```python
from build123d import *

# Parameters (mm, degrees)
SKETCH1_R           = 20
SKETCH1_R_2         = 12.5
BOSS_EXTRUDE1_DEPTH = 112
CHAMFER1_SIZE       = 1


with BuildPart() as part:
    # Sketch1 → Boss-Extrude1 (new body)
    with BuildSketch(Plane(origin=(0, 0, 0), x_dir=(1, 0, 0), z_dir=(0, 1, 0))):
        with Locations(Location((0, 0, 0), (0, 0, 270))):
            Circle(SKETCH1_R)
        with Locations(Location((0, 0, 0), (0, 0, 270))):
            Circle(SKETCH1_R_2, mode=Mode.SUBTRACT)
    extrude(amount=BOSS_EXTRUDE1_DEPTH)

    # Chamfer1
    chamfer1_edges = [part.edges().sort_by_distance(p)[0] for p in [
        (0, 0, -20),
        (0, 112, -20),
        (0, 0, -12.5),
        (0, 112, -12.5),
    ]]
    chamfer(chamfer1_edges, length=CHAMFER1_SIZE)


solid = part.part
```
Source: CAD feature listing. Evaluate the final solid. Frame: model axes, mm. Give positions to 0.01 mm unless a question says otherwise; leave off trailing zeros. Write each loop counter-clockwise with the first axis right and the second up, starting at its lowest first coordinate (ties: lowest second). Pieces come first, ordered by that corner, then holes.
1. Section query B-B (x = 0). Return the cut outline in (y, z).
2. Section query C-C (y = 67). Return the cut outline in (x, z), then the cut area to 3 significant figures.
3. Pull-direction query (Z, two-part tool) for faces 1 (the face through (3.755, 55.23, 11.923)), 2 (the face through (-19.524, 55.23, -4.336)), 3 (the face through (12.9, 112, -4.5)); classes: +Z half, -Z half, draft (parallel to the pull), parting line (faces both ways), or undercut.
4. First-contact query: pin 1 (3 mm diameter, centred on y = 55.5, z = 5, fed in from -X); pin 2 (12 mm diameter, centred on x = 4.5, z = -12, fed in from +Y); pin 3 (10 mm diameter, centred on x = -11.5, y = 97.5, fed in from +Z); pin 4 (8 mm diameter, centred on y = 37, z = -1, fed in from -X). Flat tips, straight axial feed; report the tip coordinate or a pass-through.
5. Section query A-A (z = 0). Return the cut outline in (x, y), then the cut area to 3 significant figures.
6. Material intervals for line 1 along X through (y, z) = (27, 0); line 2 along Z through (x, y) = (7, 25) (3 decimals); line 3 along Z through (x, y) = (-9, 99.5), sorted ascending.
Output values:
1. outline: (0, -19) - (1, -20) - (111, -20) - (112, -19) - (112, -13.5) - (111, -12.5) - (1, -12.5) - (0, -13.5) - close; (0, 13.5) - (1, 12.5) - (111, 12.5) - (112, 13.5) - (112, 19) - (111, 20) - (1, 20) - (0, 19) - close
2. outline: circle Ø40 at (0, 0); hole circle Ø25 at (0, 0)
2. area: 766 mm2
3. face 1: undercut
3. face 2: parting line
3. face 3: draft
4. pin 1: stops at x = -19.69
4. pin 2: stops at y = 112
4. pin 3: stops at z = 18.91
4. pin 4: stops at x = -20
5. outline: (-20, 1) - (-19, 0) - (-13.5, 0) - (-12.5, 1) - (-12.5, 111) - (-13.5, 112) - (-19, 112) - (-20, 111) - close; (12.5, 1) - (13.5, 0) - (19, 0) - (20, 1) - (20, 111) - (19, 112) - (13.5, 112) - (12.5, 111) - close
5. area: 1,680 mm2
6. line 1: x = -20 to -12.5, 12.5 to 20
6. line 2: z = -18.735 to -10.356, 10.356 to 18.735
6. line 3: z = -17.86 to -8.67, 8.67 to 17.86
